Verification items for the finished model (mm, model axes). Face numbers are marked on the shaded views. A direction names the side the tool comes from. Coordinates: 2 decimals unless noted, no trailing zeros. Write each loop counter-clockwise with the first axis right and the second up, starting at its lowest first coordinate (ties: lowest second). Pieces come first, ordered by that corner, then holes. Notation, with made-up numbers: (-7.75, -36) - (34.25, -36) arc R23 cw to (34.25, 0) - close; hole circle Ø6 at (25, -8). An arc over 180 degrees is marked (long way). Use one line per item in the form item = value. Start each with the question number.
(1) Sectioned sample at D-D (z = 6.25). Record the cut outline in (x, y).
(2) Sectioned sample at A-A (x = 0). Record the cut outline in (y, z), and give its area (3 significant figures).
(3) Tool access check on the marked faces 1, 2 and 3. Record the directions out of +Z, -Z, +X, -X, +Y, -Y that give a thin tool (end or side, any length) a straight path to the whole face; none if there is none.
(4) Material ranges on line 1 (X direction, y = -21.5, z = 0); line 2 (Y direction, x = 1, z = 7); line 3 (Y direction, x = -23, z = 1.25), recorded low to high. Write a range as [from, to].
(5) Gauge pin test, flat ends, axial feed: pin 1 Ø3 at (x, z) = (-11.5, -4) entering from +Y; pin 2 Ø2 at (x, z) = (-28, -1.5) entering from +Y; pin 3 Ø12 at (x, z) = (-24, 1) entering from -Y. Record the tip position at first contact, or that the pin passes through.
(6) Mould release check, pull along Z, two halves, no side actions. Record for the marked faces 4, 5 and 6: released by +Z, released by -Z, zero draft, split by the parting line, or undercut.
(7) Sectioned sample at B-B (z = 1). Record the cut outline in (x, y), and give its area (3 significant figures).
(8) Sectioned sample at C-C (y = 7). Record the cut outline in (x, z).
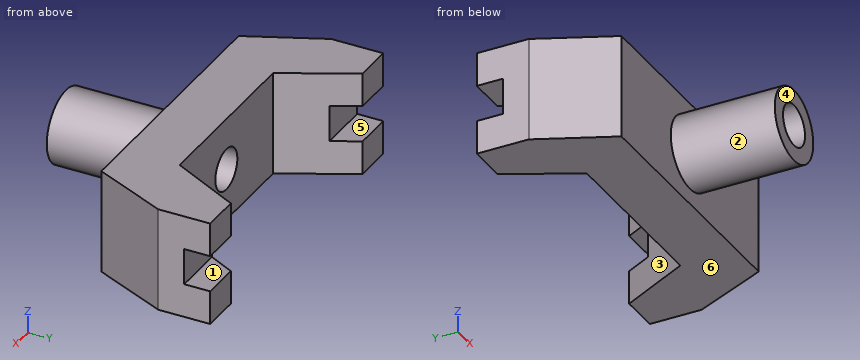
from build123d import *

# Parameters (mm, degrees)
YOKE_BODY_DEPTH      = 10
ARM_SLOTS_DEPTH      = 66.209374322
POST_SEAT_SKETCH_R   = 4
POST_SEAT_CUT_DEPTH  = 20
PIVOT_POST_SKETCH_R  = 7
PIVOT_POST_DEPTH     = 20
CENTRE_HOLE_SKETCH_R = 4
CENTRE_HOLE_DEPTH    = 46.209194984


with BuildPart() as part:
    # Yoke Profile Sketch → Yoke Body (new, symmetric)
    with BuildSketch(Plane.XY):
        Polygon((0, 0), (17, 0), (24, 13.537448042), (31.5, 13.537448042), (31.5, 3.537448042), (25, -10.848359941), (-25, -10.848359941), (-31.5, 3.537448042), (-31.5, 13.537448042), (-24, 13.537448042), (-17, 0), align=None)
    extrude(amount=YOKE_BODY_DEPTH, both=True)

    # Arm Slots Sketch → Arm Slots (cut, through all)
    with BuildSketch(Plane.ZY.offset(31.5)):
        Polygon((0, 13.537448042), (3.5, 13.537448042), (3.5, 8.537448042), (-3.5, 8.537448042), (-3.5, 13.537448042), align=None)
    extrude(amount=-ARM_SLOTS_DEPTH, mode=Mode.SUBTRACT)

    # Post Seat Sketch → Post Seat Cut (cut)
    with BuildSketch(Plane(origin=(0, 0, 0), x_dir=(1, 0, 0), z_dir=(0, 1, 0))):
        with Locations(Location((0, 0, 0), (0, 0, 270))):
            Circle(POST_SEAT_SKETCH_R)
    extrude(amount=-POST_SEAT_CUT_DEPTH, mode=Mode.SUBTRACT)

    # Pivot Post Sketch → Pivot Post (add)
    with BuildSketch(Plane.XZ.offset(10.848359941)):
        with Locations(Location((0, 0, 0), (0, 0, 90))):
            Circle(PIVOT_POST_SKETCH_R)
    extrude(amount=PIVOT_POST_DEPTH)

    # Centre Hole Sketch → Centre Hole (cut, through all)
    with BuildSketch(Plane(origin=(0, 0, 0), x_dir=(1, 0, 0), z_dir=(0, 1, 0))):
        with Locations(Location((0, 0, 0), (0, 0, 270))):
            Circle(CENTRE_HOLE_SKETCH_R)
    extrude(amount=-CENTRE_HOLE_DEPTH, mode=Mode.SUBTRACT)


solid = part.part
Answers below:
q1.outline = (-31.5, 3.54) - (-25, -10.85) - (-3.15, -10.85) - (-3.15, -30.85) - (3.15, -30.85) - (3.15, -10.85) - (25, -10.85) - (31.5, 3.54) - (31.5, 13.54) - (24, 13.54) - (17, 0) - (-17, 0) - (-24, 13.54) - (-31.5, 13.54) - close
q2.outline = (-30.85, -7) - (-10.85, -7) - (-10.85, -10) - (0, -10) - (0, -4) - (-30.85, -4) - close; (-30.85, 4) - (0, 4) - (0, 10) - (-10.85, 10) - (-10.85, 7) - (-30.85, 7) - close
q2.area = 250 mm2
q3.face_1 = +X, -X, +Y
q3.face_2 = -Y
q3.face_3 = +Z, -Z, +Y
q4.line_1 = [-7, -4], [4, 7]
q4.line_2 = [-10.85, 0]
q4.line_3 = [-10.85, 8.54]
q5.pin_1 = 0
q5.pin_2 = 8.54
q5.pin_3 = -10.85
q6.face_4 = zero draft
q6.face_5 = undercut
q6.face_6 = released by -Z
q7.outline = (-31.5, 3.54) - (-25, -10.85) - (-6.93, -10.85) - (-6.93, -30.85) - (-3.87, -30.85) - (-3.87, 0) - (-17, 0) - (-21.41, 8.54) - (-31.5, 8.54) - close; (3.87, -30.85) - (6.93, -30.85) - (6.93, -10.85) - (25, -10.85) - (31.5, 3.54) - (31.5, 8.54) - (21.41, 8.54) - (17, 0) - (3.87, 0) - close
q7.area = 838 mm2
q8.outline = (-31.5, -10) - (-20.62, -10) - (-20.62, 10) - (-31.5, 10) - close; (20.62, -10) - (31.5, -10) - (31.5, 10) - (20.62, 10) - close
